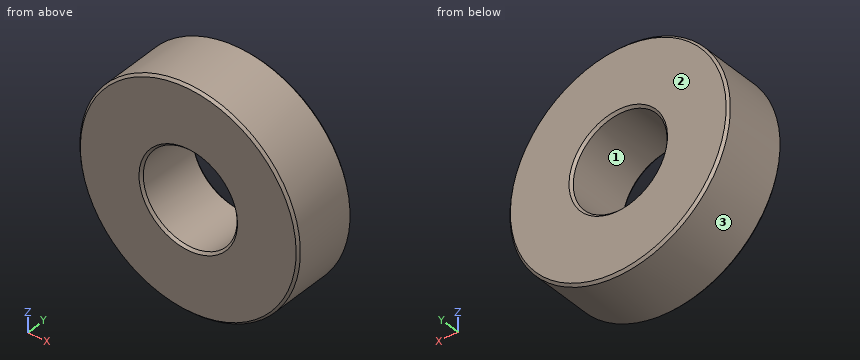
from build123d import *

# Parameters (mm, degrees)
SKETCH_1_R      = 23.5
SKETCH_1_R_2    = 10
EXTRUDE_1_DEPTH = 14
CHAMFER_1_SIZE  = 0.5


with BuildPart() as part:
    # 草图1 → 拉伸1 (new body)
    with BuildSketch(Plane(origin=(0, 0, 0), x_dir=(1, 0, 0), z_dir=(0, 1, 0))):
        with Locations(Location((0, 0, 0), (0, 0, 270))):
            Circle(SKETCH_1_R)
        with Locations(Location((0, 0, 0), (0, 0, 270))):
            Circle(SKETCH_1_R_2, mode=Mode.SUBTRACT)
    extrude(amount=EXTRUDE_1_DEPTH)

    # 倒角1
    chamfer_1_edges = [part.edges().sort_by_distance(p)[0] for p in [
        (0, 0, -23.5),
        (0, 14, -23.5),
        (0, 0, -10),
        (0, 14, -10),
    ]]
    chamfer(chamfer_1_edges, length=CHAMFER_1_SIZE)


solid = part.part
Design review of the part built by this model. Coordinates are the model's own, in mm. Face numbers are marked on the shaded views. Coordinates: 2 decimals unless noted, no trailing zeros. Loops run counter-clockwise (first coordinate to the right, second up) from the corner with the lowest first, then second, coordinate; pieces in that order, holes last. Notation, with made-up numbers: M -22,-27 L 4,-27 A22 cw 4,0 Z; hole C 26.5,-21.5 d6. An arc over 180 degrees is marked long. Use one line per item in the form item = value.
(1) Clearance check with flat-ended pins moving along their axes: P1, Ø5, axis at y = 3.5, z = -5, coming from the -X side; P2, Ø5, axis at x = 8, y = 11, coming from the +Z side; P3, Ø1, axis at x = 0.5, y = 5.5, coming from the +Z side; P4, Ø8, axis at y = 6, z = -14.5, coming from the +X side. State where each tip first meets the part, or that it passes through.
Return value:
P1 = -23.37
P2 = 22.85
P3 = 23.5
P4 = 21.02
(2) Draft analysis for pull direction Z (two halves, no side actions). For the marked faces 1, 2 and 3, state which applies: pulls with the +Z half, pulls with the -Z half, needs draft (parallel to the pull), parting line crosses it, or undercut.
Return value:
face_1 = undercut
face_2 = needs draft
face_3 = parting line crosses it
(3) For line 1 along X through (y, z) = (4.25, 0); line 2 along Z through (x, y) = (0.5, 12.25); line 3 along X through (y, z) = (7.5, -7.5), list the stretches that pass through material, from the lowest coordinate up. Write a range as from..to.
Return value:
line_1 = -23.5..-10, 10..23.5
line_2 = -23.49..-9.99, 9.99..23.49
line_3 = -22.27..-6.61, 6.61..22.27
(4) Consider section B-B (x = 0). Write out the cut boundary in (y, z).
Return value:
outline = M 0,-23 L 0.5,-23.5 L 13.5,-23.5 L 14,-23 L 14,-10.5 L 13.5,-10 L 0.5,-10 L 0,-10.5 Z; M 0,10.5 L 0.5,10 L 13.5,10 L 14,10.5 L 14,23 L 13.5,23.5 L 0.5,23.5 L 0,23 Z
(5) Consider section C-C (y = 11.5). Write out the cut boundary in (x, z).
Return value:
outline = C 0,0 d47; hole C 0,0 d20
(6) Consider section A-A (z = 0). Write out the cut boundary in (x, y).
Return value:
outline = M -23.5,0.5 L -23,0 L -10.5,0 L -10,0.5 L -10,13.5 L -10.5,14 L -23,14 L -23.5,13.5 Z; M 10,0.5 L 10.5,0 L 23,0 L 23.5,0.5 L 23.5,13.5 L 23,14 L 10.5,14 L 10,13.5 Z
